from build123d import *

# Parameters (mm, degrees)
BASE_EXTRUDE_DEPTH      = 0.5
BASE_EXTRUDE_DEPTH_BACK = 0.5
SKETCH1_R               = 0.85


with BuildPart() as part:
    # Sketch1 → Base-Extrude (new, two sides: drawn at the far end of the back side and taken through both)
    with BuildSketch(Plane.XY.offset(-BASE_EXTRUDE_DEPTH_BACK)):
        with BuildLine():
            Line((-1, -6.335364439), (-1, -9.766370259))
            ThreePointArc((-1, -9.766370259), (-3.028831825, -9.315828269), (-4.908022896, -8.428254284))
            ThreePointArc((-4.908022896, -8.428254284), (-4.968516352, -8.37034995), (-5, -8.292753881))
            Line((-5, -8.292753881), (-5.605979842, -4.856071421))
            ThreePointArc((-5.605979842, -4.856071421), (-5.643449504, -4.735447058), (-5.709951634, -4.628061401))
            ThreePointArc((-5.709951634, -4.628061401), (0, 7.35), (5.709951634, -4.628061401))
            ThreePointArc((5.709951634, -4.628061401), (5.643449504, -4.735447058), (5.605979842, -4.856071421))
            Line((5.605979842, -4.856071421), (5, -8.292753881))
            ThreePointArc((5, -8.292753881), (4.968516352, -8.37034995), (4.908022896, -8.428254284))
            ThreePointArc((4.908022896, -8.428254284), (3.028831825, -9.315828269), (1, -9.766370259))
            Line((1, -9.766370259), (1, -6.335364439))
            ThreePointArc((1, -6.335364439), (0, 5.48), (-1, -6.335364439))
        make_face()
        with Locations((-3, -7.561544261)):
            Circle(SKETCH1_R, mode=Mode.SUBTRACT)
        with Locations(Location((3, -7.561544261, 0), (0, 0, 180))):
            Circle(SKETCH1_R, mode=Mode.SUBTRACT)
    extrude(amount=BASE_EXTRUDE_DEPTH + BASE_EXTRUDE_DEPTH_BACK)


solid = part.part
For this review, take the finished solid that the model builds, in its own axes (mm). A direction names the side the tool comes from. Give positions to 0.01 mm unless a question says otherwise; leave off trailing zeros. Loops run counter-clockwise (first coordinate to the right, second up) from the corner with the lowest first, then second, coordinate; pieces in that order, holes last.
Item 1: Take a section at B-B, the plane x = -2.5. State the section outline as (y, z) points, and give its area (3 significant figures).
Item 2: Draft analysis for pull direction Y (two halves, no side actions). For faces 1 (the cylindrical face through (3.111, -8.404, -0.007)), 2 (the flat face through (1, -8, 0)), 3 (the cylindrical face through (3.056, -9.306, -0.007)), 4 (the cylindrical face through (0.248, 5.475, -0.007)), state which applies: +Y half, -Y half, draft (parallel to the pull), parting line (faces both ways), or undercut.
Item 3: For line 1 along Y through (x, z) = (3, -0.2); line 2 along Y through (x, z) = (-3.5, -0.15); line 3 along X through (y, z) = (0.25, 0.4), list the stretches that pass through material, from the lowest coordinate up.
Item 4: Take a section at D-D, the plane x = 0. State the section outline as (y, z) points, and give its area (3 significant figures).
Item 5: Insertion check: pin 1 (0.5 mm diameter, centred on y = -8.5, z = 0, fed in from -X). The pin has a flat end and moves straight along its axis. Give the tip position at first contact, or say it passes through.
Item 6: Tool access review of faces 5 (the flat face through (-1, -8, 0)), 6 (the flat face through (-3, -6, -0.5)): name each direction out of +Z, -Z, +X, -X, +Y, -Y from which nothing blocks a thin tool from reaching the whole face with its end or side.
Item 7: Take a section at C-C, the plane y = 0. State the section outline as (x, z) points.
Item 8: Take a section at A-A, the plane y = -8. State the section outline as (x, z) points.
Calculated:
1. outline: (-9.48, -0.5) - (-8.25, -0.5) - (-8.25, 0.5) - (-9.48, 0.5) - close; (-6.87, -0.5) - (-5.87, -0.5) - (-5.87, 0.5) - (-6.87, 0.5) - close; (4.93, -0.5) - (6.91, -0.5) - (6.91, 0.5) - (4.93, 0.5) - close
1. area: 4.22 mm2
2. face 1: undercut
2. face 2: draft
2. face 3: -Y half
2. face 4: undercut
3. line 1: y = -9.33 to -8.41, -6.71 to -5.61, 4.67 to 6.71
3. line 2: y = -9.14 to -8.25, -6.87 to -5.28, 4.34 to 6.46
3. line 3: x = -7.35 to -5.91, 5.91 to 7.35
4. outline: (5.48, -0.5) - (7.35, -0.5) - (7.35, 0.5) - (5.48, 0.5) - close
4. area: 1.87 mm2
5. pin 1: stops at x = -5.01
6. face 5: +Z, -Z, -Y
6. face 6: -Z, +X, -X, +Y, -Y
7. outline: (-7.35, -0.5) - (-5.93, -0.5) - (-5.93, 0.5) - (-7.35, 0.5) - close; (5.93, -0.5) - (7.35, -0.5) - (7.35, 0.5) - (5.93, 0.5) - close
8. outline: (-5.05, -0.5) - (-3.73, -0.5) - (-3.73, 0.5) - (-5.05, 0.5) - close; (-2.27, -0.5) - (-1, -0.5) - (-1, 0.5) - (-2.27, 0.5) - close; (1, -0.5) - (2.27, -0.5) - (2.27, 0.5) - (1, 0.5) - close; (3.73, -0.5) - (5.05, -0.5) - (5.05, 0.5) - (3.73, 0.5) - close
